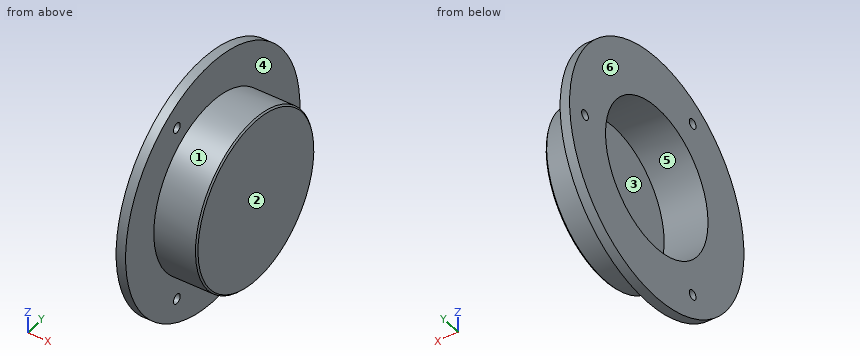
```python
from build123d import *

# Parameters (mm, degrees)
HOLE_WIZARD_M6_1_D = 6.6
CHAMFER_1_SIZE     = 1


with BuildPart() as part:
    # 草图2 → 旋转1 (revolve)
    with BuildSketch(Plane.XY, mode=Mode.PRIVATE) as revolve_1_sk:
        Polygon((30, 0), (30, 50), (0, 50), (0, 85), (6.5, 85), (6.5, 57.5), (36, 57.5), (36, 0), align=None)
    revolve(revolve_1_sk.sketch.rotate(Axis((0, 0, 0), (1, 0, 0)), 90), axis=Axis((0, 0, 0), (1, 0, 0)))

    # M6 间隙孔1 (through all)
    with Locations(Plane(origin=(6.5, 0, 0), x_dir=(0, 0, -1), z_dir=(1, 0, 0))):
        with Locations((-60.621778265, -35), (0, 70), (60.621778265, -35)):
            Hole(HOLE_WIZARD_M6_1_D / 2)

    # 倒角1
    chamfer_1_edges = [part.edges().sort_by_distance(p)[0] for p in [
        (36, 0, -57.5),
    ]]
    chamfer(chamfer_1_edges, length=CHAMFER_1_SIZE)


solid = part.part
```
Geometry check sheet. Reference: the model listing, model coordinates, mm. Face numbers are marked on the shaded views. A direction names the side the tool comes from. Round coordinates to 2 decimals unless told otherwise and drop trailing zeros. Order: outer loops, then holes, each group sorted by start corner. A loop starts at its lowest first (then second) coordinate and runs counter-clockwise, first axis right, second up. Notation, with made-up numbers: (-20, -9) - (13, -9) arc R14 ccw to (13, 0) - close; hole circle Ø5 at (-16.5, 51.25). An arc over 180 degrees is marked (long way). Use a Markdown table: item, result. Add a question column.
1) Section check C-C (y = 70). Record the cut outline in (x, z), then the cut area to 3 significant figures.
2) Gauge pin test, flat ends, axial feed: P1, Ø1, axis at x = 14.5, z = 33, coming from the +Y side; P2, Ø12, axis at x = 15.5, z = 20.5, coming from the +Y side; P3, Ø12, axis at x = 18, z = 16.5, coming from the -Y side. Record the tip position at first contact, or that the pin passes through.
3) Section check B-B (y = 0). Record the cut outline in (x, z), then the cut area to 3 significant figures.
4) Section check D-D (x = 27). Record the cut outline in (y, z).
5) Mould release check, pull along Z, two halves, no side actions. Record for the marked faces 1, 2 and 3: released by +Z, released by -Z, zero draft, split by the parting line, or undercut.
6) Section check A-A (z = 0). Record the cut outline in (x, y), then the cut area to 3 significant figures.
7) Set-up check for the marked faces 4, 5 and 6: record each of +Z, -Z, +X, -X, +Y, -Y from which the full face is reachable in a straight line by a thin tool's end or side.
8) Thickness scan on line 1 along Y through (x, z) = (4.5, 0); line 2 along Y through (x, z) = (28, -1); line 3 along X through (y, z) = (-8.5, -69). Record the ranges inside material, lowest first.
Established:
| question | item | result |
|---|---|---|
| 1 | outline | (0, -48.22) - (6.5, -48.22) - (6.5, -3.3) - (0, -3.3) - close; (0, 3.3) - (6.5, 3.3) - (6.5, 48.22) - (0, 48.22) - close |
| 1 | area | 584 mm2 |
| 2 | P1 | y = 47.43 |
| 2 | P2 | y = 55.64 |
| 2 | P3 | y = -56.53 |
| 3 | outline | (0, -85) - (6.5, -85) - (6.5, -57.5) - (35, -57.5) - (36, -56.5) - (36, 56.5) - (35, 57.5) - (6.5, 57.5) - (6.5, 85) - (0, 85) - (0, 50) - (30, 50) - (30, -50) - (0, -50) - close |
| 3 | area | 1,500 mm2 |
| 4 | outline | circle Ø115 at (0, 0); hole circle Ø100 at (0, 0) |
| 5 | face 1 | split by the parting line |
| 5 | face 2 | zero draft |
| 5 | face 3 | undercut |
| 6 | outline | (0, -85) - (6.5, -85) - (6.5, -57.5) - (35, -57.5) - (36, -56.5) - (36, 56.5) - (35, 57.5) - (6.5, 57.5) - (6.5, 66.7) - (0, 66.7) - (0, 50) - (30, 50) - (30, -50) - (0, -50) - close; (0, 73.3) - (6.5, 73.3) - (6.5, 85) - (0, 85) - close |
| 6 | area | 1,450 mm2 |
| 7 | face 4 | +X |
| 7 | face 5 | -X |
| 7 | face 6 | +Z, -Z, -X, +Y, -Y |
| 8 | line 1 | -85 to -50, 50 to 66.7, 73.3 to 85 |
| 8 | line 2 | -57.49 to -49.99, 49.99 to 57.49 |
| 8 | line 3 | 0 to 6.5 |
